from build123d import *

# Parameters (mm, degrees)
SKETCH_1_W          = 645
SKETCH_1_H          = 900
EXTRUDE_1_DEPTH     = 594.5
SKETCH_2_W          = 605
SKETCH_2_H          = 554.5
SKETCH_2_W_2        = 595
SKETCH_2_H_2        = 544.5
CUT_EXTRUDE_1_DEPTH = 10
SKETCH_3_R          = 20
EXTRUDE_2_DEPTH     = 5
SKETCH_4_W          = 9.930578971
SKETCH_4_H          = 24.659600502
CUT_EXTRUDE_2_DEPTH = 5
SKETCH_5_W          = 605
SKETCH_5_H          = 554.5
SKETCH_5_W_2        = 595
SKETCH_5_H_2        = 544.5
CUT_EXTRUDE_3_DEPTH = 10
SKETCH_6_R          = 20
EXTRUDE_3_DEPTH     = 5
SKETCH_7_W          = 13.385113247
SKETCH_7_H          = 26.065674485
CUT_EXTRUDE_4_DEPTH = 5


with BuildPart() as part:
    # 草图1 → 凸台-拉伸1 (new body)
    with BuildSketch(Plane.XY):
        Rectangle(SKETCH_1_W, SKETCH_1_H)
    extrude(amount=EXTRUDE_1_DEPTH)

    # 草图2 → 切除-拉伸1 (cut)
    with BuildSketch(Plane.XZ.offset(450)):
        with Locations((0, 297.25)):
            Rectangle(SKETCH_2_W, SKETCH_2_H)
        with Locations((0, 297.25)):
            Rectangle(SKETCH_2_W_2, SKETCH_2_H_2, mode=Mode.SUBTRACT)
    extrude(amount=-CUT_EXTRUDE_1_DEPTH, mode=Mode.SUBTRACT)

    # 草图3 → 凸台-拉伸2 (add)
    with BuildSketch(Plane.XZ.offset(450)):
        with Locations(Location((263.592324158, 304.229859051, 0), (0, 0, 90))):
            Circle(SKETCH_3_R)
    extrude(amount=EXTRUDE_2_DEPTH)

    # 草图4 → 切除-拉伸2 (cut)
    with BuildSketch(Plane.XZ.offset(455)):
        with Locations((263.592324158, 304.229859051)):
            Rectangle(SKETCH_4_W, SKETCH_4_H)
    extrude(amount=-CUT_EXTRUDE_2_DEPTH, mode=Mode.SUBTRACT)

    # 草图5 → 切除-拉伸3 (cut)
    with BuildSketch(Plane(origin=(0, 450, 0), x_dir=(1, 0, 0), z_dir=(0, 1, 0))):
        with Locations((0, -297.25)):
            Rectangle(SKETCH_5_W, SKETCH_5_H)
        with Locations((0, -297.25)):
            Rectangle(SKETCH_5_W_2, SKETCH_5_H_2, mode=Mode.SUBTRACT)
    extrude(amount=-CUT_EXTRUDE_3_DEPTH, mode=Mode.SUBTRACT)

    # 草图6 → 凸台-拉伸3 (add)
    with BuildSketch(Plane(origin=(0, 450, 0), x_dir=(1, 0, 0), z_dir=(0, 1, 0))):
        with Locations(Location((-261.325922866, -300.206175598, 0), (0, 0, 90))):
            Circle(SKETCH_6_R)
    extrude(amount=EXTRUDE_3_DEPTH)

    # 草图7 → 切除-拉伸4 (cut)
    with BuildSketch(Plane(origin=(0, 455, 0), x_dir=(1, 0, 0), z_dir=(0, 1, 0))):
        with Locations((-261.325922867, -300.206175599)):
            Rectangle(SKETCH_7_W, SKETCH_7_H)
    extrude(amount=-CUT_EXTRUDE_4_DEPTH, mode=Mode.SUBTRACT)


solid = part.part
Read the model definition and answer for the solid it produces. Units are mm, in the model's axes. A direction names the side the tool comes from. Round coordinates to 2 decimals unless told otherwise and drop trailing zeros.
Q1. Consider probe 1 along Y at (x, z) = (43.5, 545.5). Determine where the line is inside the solid, lowest interval first.
Q2. Which of the six approach directions +Z, -Z, +X, -X, +Y, -Y give full straight-line access (tool end or side, diameter ignored) to faces 1 (the face through (271.252, -452.465, 322.705)), 2 (the face through (-253.67, 452.46, 281.73)), 3 (the face through (-5, 6, 594.5))?
Q3. Each of these flat-tipped pins is pushed along its axis until it touches: pin 1 (8 mm diameter, centred on x = -84, z = 181.5, fed in from +Y); pin 2 (8 mm diameter, centred on x = -38, z = 226, fed in from -Y); pin 3 (1.5 mm diameter, centred on y = -452.5, z = 301.5, fed in from -X). Where does it stop, or does it pass through?
Output:
1. probe 1: y = -450 to 450
2. face 1: -Y
2. face 2: +Y
2. face 3: +Z, +X, -X, +Y, -Y
3. pin 1: stops at y = 450
3. pin 2: stops at y = -450
3. pin 3: stops at x = 243.69
